Source: CAD feature listing. Evaluate the final solid. Frame: model axes, mm. Give positions to 0.01 mm unless a question says otherwise; leave off trailing zeros. Order: outer loops, then holes, each group sorted by start corner. A loop starts at its lowest first (then second) coordinate and runs counter-clockwise, first axis right, second up. Notation, with made-up numbers: M 36.25,44 L 67.25,44 A20 cw 67.25,60 Z; hole C 40.5,51.5 d8. An arc over 180 degrees is marked long. Answer as a JSON object with one key per item and string values. Group by question number.
1. Section query A-A (y = 0). Output: boundary loops of the cut face in (x, z), plus the area to 3 significant figures.
2. Section query B-B (x = 0). Output: boundary loops of the cut face in (y, z), plus the area to 3 significant figures.
3. Material intervals for L1, parallel to X at y = 1, z = 3.5; L2, parallel to Y at x = 0, z = 2.3; L3, parallel to X at y = -33.5, z = 4.5, sorted ascending. Write a range as [from, to].
from build123d import *


with BuildPart() as part:
    # Sweep1: sweep along a path in Sketch1
    with BuildLine(Plane.XY) as sweep1_path:
        Line((30.251612903, 153.344481207), (627.025806452, 35.613593524))
        ThreePointArc((627.025806452, 35.613593524), (656.3, 0), (627.025806452, -35.613593524))
        Line((627.025806452, -35.613593524), (30.251612903, -153.344481207))
        ThreePointArc((30.251612903, -153.344481207), (-156.3, 0), (30.251612903, 153.344481207))
    # Sketch2 → Sweep1 (sweep)
    with BuildSketch(Plane(origin=(0, 0, 0), x_dir=(1, 0, 0), z_dir=(0, 1, 0))):
        Polygon((-156.3, 0), (-156.3, -5), (-167.8, -9), (-167.8, 4), align=None)
    sweep(path=sweep1_path.line)


solid = part.part
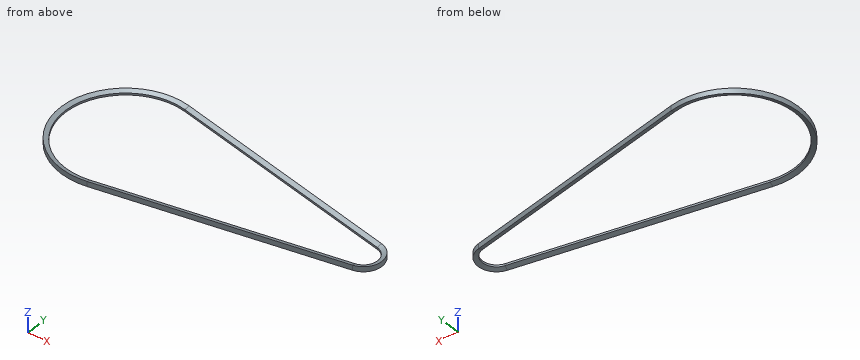
Answer sheet:
{
 "1": {"outline": "M -167.8,-4 L -156.3,0 L -156.3,5 L -167.8,9 Z; M 656.3,0 L 667.8,-4 L 667.8,9 L 656.3,5 Z", "area": "207 mm^2"},
 "2": {"outline": "M -167.8,-4 L -156.3,0 L -156.3,5 L -167.8,9 Z; M 156.3,0 L 167.8,-4 L 167.8,9 L 156.3,5 Z", "area": "207 mm^2"},
 "3": {"L1": "[-167.8, -156.3], [656.29, 667.79]", "L2": "[-167.8, -156.3], [156.3, 167.8]", "L3": "[-164.42, -152.67], [633.98, 654.1]"}
}
